Geometry check sheet. Reference: the model listing, model coordinates, mm. A direction names the side the tool comes from. Give positions to 0.01 mm unless a question says otherwise; leave off trailing zeros. Write each loop counter-clockwise with the first axis right and the second up, starting at its lowest first coordinate (ties: lowest second). Pieces come first, ordered by that corner, then holes.
(1) Depth check by flat-ended pin: P1, Ø4, axis at x = -165, z = 284.5, coming from the -Y side; P2, Ø3, axis at y = -339.5, z = 284.5, coming from the +X side; P3, Ø10, axis at y = -220, z = 214, coming from the +X side. Enter the tip coordinate at first touch or a pass-through.
(2) Thickness scan on line 1 along X through (y, z) = (-34, 254.5); line 2 along Z through (x, y) = (-4.5, -1427); line 3 along Z through (x, y) = (-155, 65). Record the ranges inside material, lowest first.
(3) Cross-section at A-A (z = 286.5). Record the boundary of the cut face in (x, y), and give its area (3 significant figures).
(4) Cross-section at D-D (z = 63). Record the boundary of the cut face in (x, y).
(5) Mould release check, pull along X, two halves, no side actions. Record for faces 5 (the flat face through (-3, -1180, 250)), 6 (the flat face through (-2, -150, 301)), 7 (the flat face through (-175, -3, 223)): +X half, -X half, draft (parallel to the pull), parting line (faces both ways), or undercut.
(6) Tool access check on faces 1 (the flat face through (-2, 2, 250)), 2 (the flat face through (-225, -1200, 123)), 3 (the flat face through (-2, -3, 100)), 4 (the flat face through (175, 3, 223)). Record the directions out of +Z, -Z, +X, -X, +Y, -Y that give a thin tool (end or side, any length) a straight path to the whole face; none if there is none.
(7) Cross-section at C-C (y = -113). Record the boundary of the cut face in (x, z).
(8) Cross-section at B-B (x = 22). Record the boundary of the cut face in (y, z), and give its area (4 significant figures).
```python
from build123d import *

# Parameters (mm, degrees)
BOSS_EXTRUDE1_DEPTH = 350
CUT_EXTRUDE1_DEPTH  = 2023.028684267
SKETCH4_W           = 250
SKETCH4_H           = 300
CUT_EXTRUDE2_DEPTH  = 100


with BuildPart() as part:
    # Sketch2 → Boss-Extrude1 (new body)
    with BuildSketch(Plane.XY):
        Polygon((-175, 190), (175, 190), (175, -190), (225, -440), (225, -1940), (-225, -1940), (-225, -440), (-175, -190), align=None)
    extrude(amount=BOSS_EXTRUDE1_DEPTH)

    # Sketch3 → Cut-Extrude1 (cut, through all)
    with BuildSketch(Plane.ZY.offset(225)):
        Polygon((350, -190), (250, -440), (250, -1940), (350, -1940), align=None)
        Polygon((0, -440), (100, -190), (100, 190), (0, 190), align=None)
    extrude(amount=-CUT_EXTRUDE1_DEPTH, mode=Mode.SUBTRACT)

    # Sketch4 → Cut-Extrude2 (cut)
    with BuildSketch(Plane.XY.offset(350)):
        Rectangle(SKETCH4_W, SKETCH4_H)
    extrude(amount=-CUT_EXTRUDE2_DEPTH, mode=Mode.SUBTRACT)


solid = part.part
```
Reply:
1. P1: stops at y = -358.75
1. P2: stops at x = 205.2
1. P3: stops at x = 182
2. line 1: x = -175 to -125, 125 to 175
2. line 2: z = 0 to 250
2. line 3: z = 100 to 350
3. outline: (-206.75, -348.75) - (206.75, -348.75) - (175, -190) - (175, 190) - (-175, 190) - (-175, -190) - close; hole (-125, -150) - (125, -150) - (125, 150) - (-125, 150) - close
3. area: 119,000 mm2
4. outline: (-225, -1940) - (225, -1940) - (225, -440) - (193.5, -282.5) - (-193.5, -282.5) - (-225, -440) - close
5. face 5: draft
5. face 6: undercut
5. face 7: -X half
6. face 1: +Z
6. face 2: +Z, -Z, -X, +Y, -Y
6. face 3: -Z, +X, -X, +Y
6. face 4: +Z, -Z, +X, +Y
7. outline: (-175, 100) - (175, 100) - (175, 350) - (125, 350) - (125, 250) - (-125, 250) - (-125, 350) - (-175, 350) - close
8. outline: (-1940, 0) - (-440, 0) - (-190, 100) - (190, 100) - (190, 350) - (150, 350) - (150, 250) - (-150, 250) - (-150, 350) - (-190, 350) - (-440, 250) - (-1940, 250) - close
8. area: 502,500 mm2
